Could you check a few things on this drawing? It's one solid part, dimensions in mm from its lowest x, y, z. A direction names the side the tool comes from. Give positions to 0.01 mm unless a question says otherwise; leave off trailing zeros. Order: outer loops, then holes, each group sorted by start corner. A loop starts at its lowest first (then second) coordinate and runs counter-clockwise, first axis right, second up. Notation, with made-up numbers: M 32,-15 L 63,-15 A30 ccw 63,19 Z; hole C 67,-31 d11. An arc over 180 degrees is marked long. Use one line per item in the form item = value.
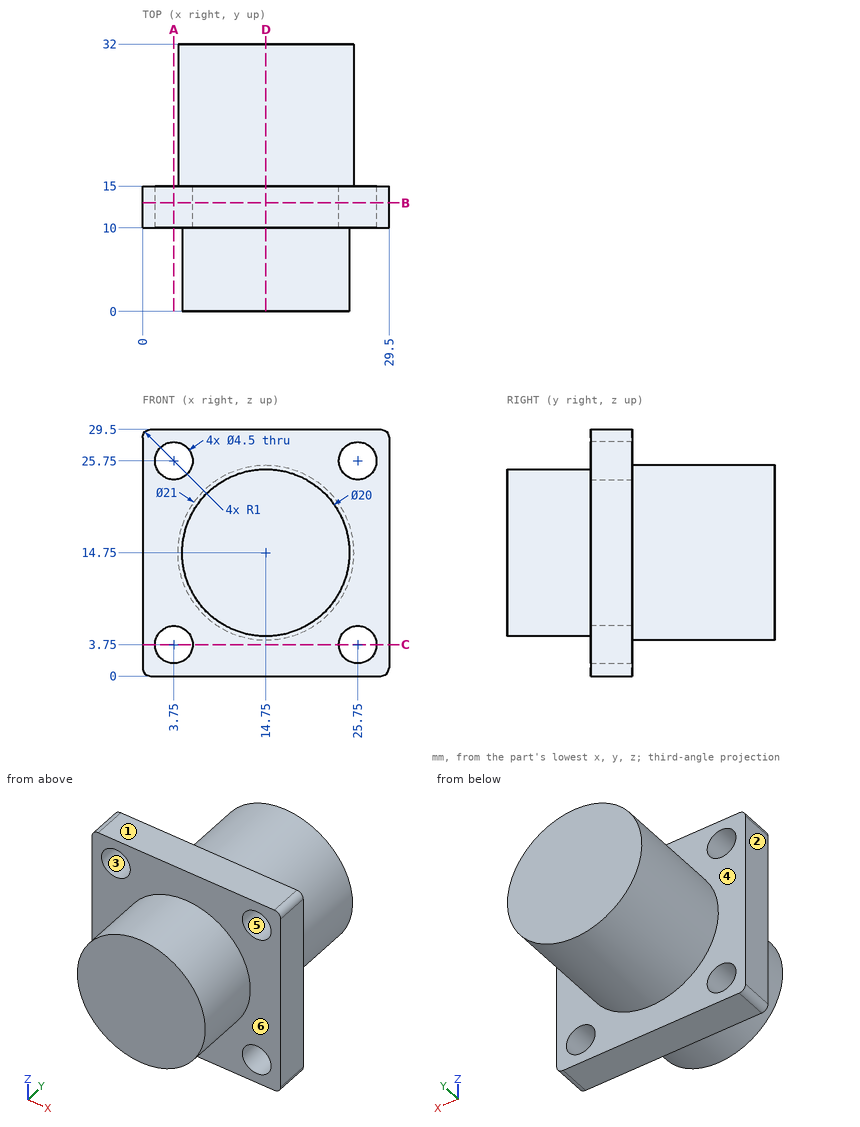
Q1. I need wall thicknesses on L1, parallel to X at y = 13.6, z = 25.75; L2, parallel to Y at x = 6.75, z = 7.25; L3, parallel to X at y = 17, z = 14.5. Which ranges of each line are inside material? Lowest first, please.
Found:
L1 = 0 to 1.5, 6 to 23.5, 28 to 29.5
L2 = 10 to 15
L3 = 4.25 to 25.25
Q2. Thinking about a two-plate mould opening in X: for the marked faces 1, 2 and 3, which applies, +X half, -X half, draft (parallel to the pull), parting line (faces both ways), or undercut?
Found:
face_1 = draft
face_2 = -X half
face_3 = undercut
Q3. On a 3-axis mill with a long thin cutter (end or side, diameter ignored), from which of +Z, -Z, +X, -X, +Y, -Y can I reach the whole of each face in a straight line? I mean the marked faces 4, 5 and 6. Say none if no direction works.
Found:
face_4 = +Y
face_5 = +Y, -Y
face_6 = -Y
Q4. I want a section at D-D on x = 14.75. Write out the boundary of the cut face in (y, z), then the cut area to 4 significant figures.
Found:
outline = M 0,4.75 L 10,4.75 L 10,0 L 15,0 L 15,4.25 L 32,4.25 L 32,25.25 L 15,25.25 L 15,29.5 L 10,29.5 L 10,24.75 L 0,24.75 Z
area = 704.5 mm²
Q5. I'm going to push flat-ended pins straight in: pin 1 Ø1 at (y, z) = (22.5, 7.5) entering from -X; pin 2 Ø7 at (x, z) = (3.75, 3.75) entering from -Y; pin 3 Ø6 at (x, z) = (25.75, 25.75) entering from +Y. Where does each tip first touch, or does it pass through?
Found:
pin_1 = 6.71
pin_2 = 10
pin_3 = 15
Q6. I want a section at A-A on x = 3.75. Write out the boundary of the cut face in (y, z), then the cut area to 4 significant figures.
Found:
outline = M 10,0 L 15,0 L 15,1.5 L 10,1.5 Z; M 10,6 L 15,6 L 15,23.5 L 10,23.5 Z; M 10,28 L 15,28 L 15,29.5 L 10,29.5 Z
area = 102.5 mm²
Q7. I want a section at C-C on z = 3.75. Write out the boundary of the cut face in (x, y).
Found:
outline = M 0,10 L 1.5,10 L 1.5,15 L 0,15 Z; M 6,10 L 23.5,10 L 23.5,15 L 6,15 Z; M 28,10 L 29.5,10 L 29.5,15 L 28,15 Z
Q8. I want a section at B-B on y = 13. Write out the boundary of the cut face in (x, z).
Found:
outline = M 0,1 A1 ccw 1,0 L 28.5,0 A1 ccw 29.5,1 L 29.5,28.5 A1 ccw 28.5,29.5 L 1,29.5 A1 ccw 0,28.5 Z; hole C 3.75,3.75 d4.5; hole C 3.75,25.75 d4.5; hole C 25.75,3.75 d4.5; hole C 25.75,25.75 d4.5
